Here's how the part is built. I have some questions about the finished solid (model axes, mm). A direction names the side the tool comes from. Round coordinates to 2 decimals unless told otherwise and drop trailing zeros. Write each loop counter-clockwise with the first axis right and the second up, starting at its lowest first coordinate (ties: lowest second). Pieces come first, ordered by that corner, then holes. Notation, with made-up numbers: M 72.25,4.25 L 79.25,4.25 A19 ccw 79.25,24.25 Z; hole C 83.5,74.5 d7. An arc over 180 degrees is marked long. Use a Markdown table: item, result. Add a question column.
```python
from build123d import *

# Parameters (mm, degrees)
U_FORK_PLATE_DEPTH      = 10
SPLIT_COLLAR_DEPTH      = 22
COLLAR_BORE_SKETCH_R    = 7.54
COLLAR_BORE_DEPTH       = 44
EYE_LUG_FRONT_SKETCH_R  = 4.525
EYE_LUG_FRONT_DEPTH     = 6
EYE_START               = -6
EYE_LUG_REAR_SKETCH_R   = 4.525
EYE_LUG_REAR_DEPTH      = 6
EYE_START_2             = -30
EYE_HOLE_SKETCH_R       = 7.54
EYE_CROSS_HOLE_DEPTH    = 30
FORK_PIN_A_SKETCH_R     = 5
FORK_PIN_A_10_DEPTH     = 6.5
FORK_PIN_B_SKETCH_R     = 5
FORK_PIN_B_10_DEPTH     = 6.5
FORK_EDGE_FILLET_R4_A_R = 4
FORK_EDGE_FILLET_R4_B_R = 4


with BuildPart() as part:
    # U-Fork Profile Sketch → U-Fork Plate (new body)
    with BuildSketch(Plane.XY):
        with BuildLine():
            ThreePointArc((19, -17.667211171), (32.551025104, -31.373310069), (37.504190816, -50))
            Line((37.504190816, -50), (37.504190816, -75))
            Line((37.504190816, -75), (31.504190816, -75))
            Line((31.504190816, -75), (31.504190816, -50))
            ThreePointArc((31.504190816, -50), (0.004190816, -18.5), (-31.495809184, -50))
            Line((-31.495809184, -50), (-31.495809184, -75))
            Line((-31.495809184, -75), (-37.495809184, -75))
            Line((-37.495809184, -75), (-37.495809184, -50))
            ThreePointArc((-37.495809184, -50), (-32.545057682, -31.377529106), (-19, -17.672136918))
            Line((-19, -17.672136918), (-19, 0))
            Line((-19, 0), (19, 0))
            Line((19, 0), (19, -17.667211171))
        make_face()
    extrude(amount=U_FORK_PLATE_DEPTH)

    # Collar Sketch → Split Collar (add, symmetric)
    with BuildSketch(Plane(origin=(0, 0, 0), x_dir=(0, 0, -1), z_dir=(1, 0, 0))):
        with BuildLine():
            Line((-7, 7.269910591), (-7, 12.338962679))
            ThreePointArc((-7, 12.338962679), (-5, -12.5), (-3, 12.338962679))
            Line((-3, 12.338962679), (-3, 7.269910591))
            ThreePointArc((-3, 7.269910591), (-5, -7.54), (-7, 7.269910591))
        make_face()
    extrude(amount=SPLIT_COLLAR_DEPTH, both=True)

    # Collar Bore Sketch → Collar Bore (cut)
    with BuildSketch(Plane(origin=(19, 0, 0), x_dir=(0, 0, -1), z_dir=(1, 0, 0))):
        with Locations((-5, 0)):
            Circle(COLLAR_BORE_SKETCH_R)
    extrude(amount=-COLLAR_BORE_DEPTH, mode=Mode.SUBTRACT)

    # Eye Lug Front Sketch → Eye Lug Front (add)
    with BuildSketch(Plane.XY.offset(7)):
        with BuildLine():
            Line((-10, 5.516178569), (10, 5.516178569))
            Line((10, 5.516178569), (10, 20.516178569))
            ThreePointArc((10, 20.516178569), (0, 30.516178569), (-10, 20.516178569))
            Line((-10, 20.516178569), (-10, 5.516178569))
        make_face()
        with Locations((0, 20.516178569)):
            Circle(EYE_LUG_FRONT_SKETCH_R, mode=Mode.SUBTRACT)
    extrude(amount=EYE_LUG_FRONT_DEPTH)

    # Eye Lug Rear Sketch → Eye Lug Rear (add)
    with BuildSketch(Plane.XY.offset(3).offset(EYE_START)):
        with BuildLine():
            Line((10, 20.516178569), (10, 5.516178569))
            Line((10, 5.516178569), (-10, 5.516178569))
            Line((-10, 5.516178569), (-10, 20.516178569))
            ThreePointArc((-10, 20.516178569), (0, 30.516178569), (10, 20.516178569))
        make_face()
        with Locations((0, 20.516178569)):
            Circle(EYE_LUG_REAR_SKETCH_R, mode=Mode.SUBTRACT)
    extrude(amount=EYE_LUG_REAR_DEPTH)

    # Eye Hole Sketch → Eye Cross Hole (cut)
    with BuildSketch(Plane.ZY.offset(10).offset(EYE_START_2)):
        with Locations((5, 0)):
            Circle(EYE_HOLE_SKETCH_R)
    extrude(amount=EYE_CROSS_HOLE_DEPTH, mode=Mode.SUBTRACT)

    # Fork Pin A Sketch → Fork Pin A Ø10 (add, symmetric)
    with BuildSketch(Plane(origin=(34.5, 0, 0), x_dir=(0, 0, -1), z_dir=(1, 0, 0))):
        with Locations((-5, -75)):
            Circle(FORK_PIN_A_SKETCH_R)
    extrude(amount=FORK_PIN_A_10_DEPTH, both=True)

    # Fork Pin B Sketch → Fork Pin B Ø10 (add, symmetric)
    with BuildSketch(Plane(origin=(-34.5, 0, 0), x_dir=(0, 0, -1), z_dir=(1, 0, 0))):
        with Locations((-5, -75)):
            Circle(FORK_PIN_B_SKETCH_R)
    extrude(amount=FORK_PIN_B_10_DEPTH, both=True)

    # Fork Edge Fillet R4 A
    fork_edge_fillet_r4_a_edges = [part.edges().sort_by_distance(p)[0] for p in [
        (19, -17.667211171, 5),
    ]]
    fillet(fork_edge_fillet_r4_a_edges, radius=FORK_EDGE_FILLET_R4_A_R)

    # Fork Edge Fillet R4 B
    fork_edge_fillet_r4_b_edges = [part.edges().sort_by_distance(p)[0] for p in [
        (-19, -17.672136918, 5),
    ]]
    fillet(fork_edge_fillet_r4_b_edges, radius=FORK_EDGE_FILLET_R4_B_R)


solid = part.part
```
Item 1: Imagine slicing it at B-B on y = 0. List the corners of the cut face in (x, z) for me.
Item 2: I need wall thicknesses on probe 1 along X at (y, z) = (-72.5, 2.25); probe 2 along Z at (x, y) = (1, 0); probe 3 along Y at (x, z) = (0, -1). Which ranges of each line are inside material? Lowest first, please. Write a range as from..to.
Item 3: Imagine slicing it at D-D on y = -21. List the corners of the cut face in (x, z) for me.
Item 4: Imagine slicing it at C-C on z = 5. List the corners of the cut face in (x, y) for me.
Item 5: Imagine slicing it at A-A on x = 0. List the corners of the cut face in (y, z) for me.
Item 6: On a 3-axis mill with a long thin cutter (end or side, diameter ignored), from which of +Z, -Z, +X, -X, +Y, -Y can I reach the whole of each face in a straight line? I mean faces 1 (the face through (0.1, 15.6, -3)), 2 (the face through (-19.46, -17.32, 5.07)), 3 (the face through (0.697, -18.508, 4.93)), 4 (the face through (-0.1, 15.6, 13)), 5 (the face through (8.5, -19.5, 10)). Say none if no direction works.
Item 7: For pin 1 Ø12 at (x, z) = (-12.5, -3) entering from +Y; pin 2 Ø5.5 at (x, y) = (0, 20.52) entering from -Z; pin 3 Ø3 at (y, z) = (17, 11) entering from -X; pin 4 Ø5 at (y, z) = (-60, 3) entering from -X, each with a flat end and sliding along its axis, tell me the tip position at first contact or that it passes through.
The answers:
| question | item | result |
|---|---|---|
| 1 | outline | M -22,-7.5 L 22,-7.5 L 22,-2.54 L -22,-2.54 Z; M -22,12.54 L 22,12.54 L 22,17.5 L -22,17.5 Z |
| 2 | probe 1 | -41..-28, 28..41 |
| 2 | probe 2 | -7.5..-2.54, 12.54..17.5 |
| 2 | probe 3 | -10.97..-4.57, 4.57..15.99, 25.04..30.52 |
| 3 | outline | M -23.77,0 L -12.29,0 L -12.29,10 L -23.77,10 Z; M 12.3,0 L 23.78,0 L 23.78,10 L 12.3,10 Z |
| 4 | outline | M -41,-80 L -28,-80 L -28,-70 L -31.5,-70 L -31.5,-50 A31.5 cw 31.5,-50 L 31.5,-70 L 28,-70 L 28,-80 L 41,-80 L 41,-70 L 37.5,-70 L 37.5,-50 A37.5 ccw 20.78,-18.78 A4 cw 19,-15.45 L 19,-12.5 L 22,-12.5 L 22,-7.54 L -22,-7.54 L -22,-12.5 L -19,-12.5 L -19,-15.46 A4 cw -20.78,-18.79 A37.5 ccw -37.5,-50 L -37.5,-70 L -41,-70 Z |
| 5 | outline | M -18.5,0 L -11.46,0 A12.5 ccw 9.6,-3 L 15.99,-3 L 15.99,3 L 7.27,3 A7.54 cw long 7.27,7 L 15.99,7 L 15.99,13 L 9.6,13 A12.5 ccw -11.46,10 L -18.5,10 Z; M 25.04,-3 L 30.52,-3 L 30.52,3 L 25.04,3 Z; M 25.04,7 L 30.52,7 L 30.52,13 L 25.04,13 Z |
| 6 | face 1 | -Z, +X, -X, +Y |
| 6 | face 2 | +Z, -Z, -X |
| 6 | face 3 | +Z, -Z |
| 6 | face 4 | +Z, +X, -X, +Y |
| 6 | face 5 | +Z, +X, -X, -Y |
| 7 | pin 1 | y = 28.12 |
| 7 | pin 2 | through |
| 7 | pin 3 | x = -10 |
| 7 | pin 4 | x = -37.5 |
